```python
from build123d import *

# Parameters (mm, degrees)
SKETCH_1_W                = 499
SKETCH_1_H                = 50
EXTRUDE_1_DEPTH           = 30
CHAMFER_1_SIZE            = 3
HOLE_WIZARD_M6_1_D        = 5
HOLE_WIZARD_M6_1_DEPTH    = 15
HOLE_WIZARD_M6_1_TIP      = 1.502151548
HOLE_WIZARD_1_D           = 6.6
HOLE_WIZARD_1_DEPTH       = 30
HOLE_WIZARD_1_CBORE_D     = 11
HOLE_WIZARD_1_CBORE_DEPTH = 6.8
HOLE_WIZARD_1_TIP         = 1.982840043


with BuildPart() as part:
    # 草图1 → 凸台-拉伸1 (new body)
    with BuildSketch(Plane(origin=(0, 0, 0), x_dir=(1, 0, 0), z_dir=(0, 1, 0))):
        Rectangle(SKETCH_1_W, SKETCH_1_H)
    extrude(amount=EXTRUDE_1_DEPTH)

    # 倒角1
    chamfer_1_edges = [part.edges().sort_by_distance(p)[0] for p in [
        (249.5, 15, 25),
        (-249.5, 15, 25),
        (-249.5, 15, -25),
        (249.5, 15, -25),
    ]]
    chamfer(chamfer_1_edges, length=CHAMFER_1_SIZE)

    # M6 螺纹孔1
    with Locations(Plane(origin=(0, 30, 0), x_dir=(1, 0, 0), z_dir=(0, 1, 0))):
        with Locations((199.5, 0), (139.5, 0), (79.5, 0), (19.5, 0), (-40.5, 0), (-100.5, 0), (-160.5, 0), (-220.5, 0)):
            Hole(HOLE_WIZARD_M6_1_D / 2, depth=HOLE_WIZARD_M6_1_DEPTH)
            with Locations((0, 0, -(HOLE_WIZARD_M6_1_DEPTH + HOLE_WIZARD_M6_1_TIP / 2))):  # 118° drill point
                Cone(0, HOLE_WIZARD_M6_1_D / 2, HOLE_WIZARD_M6_1_TIP, mode=Mode.SUBTRACT)

    # 打孔尺寸(%根据)内六角圆柱头螺钉的类型1
    with Locations(Plane(origin=(0, 30, 0), x_dir=(1, 0, 0), z_dir=(0, 1, 0))):
        with Locations((169.5, 0), (49.5, 0), (-70.5, 0), (-190.5, 0)):
            CounterBoreHole(HOLE_WIZARD_1_D / 2, HOLE_WIZARD_1_CBORE_D / 2, HOLE_WIZARD_1_CBORE_DEPTH, depth=HOLE_WIZARD_1_DEPTH)
            with Locations((0, 0, -(HOLE_WIZARD_1_DEPTH + HOLE_WIZARD_1_TIP / 2))):  # 118° drill point
                Cone(0, HOLE_WIZARD_1_D / 2, HOLE_WIZARD_1_TIP, mode=Mode.SUBTRACT)


solid = part.part
```
CAD build for the part. Positions are in the model's coordinates, mm. A direction names the side the tool comes from. Coordinates: 2 decimals unless noted, no trailing zeros. Use a Markdown table: item, result. Add a question column.
(1) Which spindle directions (+Z, -Z, +X, -X, +Y, -Y) get a long thin tool onto all of the face, cutting with end or side? Do faces 1 (the face through (-3, 30, 0)), 2 (the face through (-191, 23.2, 4)). Say none if no direction does.
(2) Drill centre lines: line 1 along Z through (x, y) = (139.5, 23); line 2 along Z through (x, y) = (-190.5, 5). Where is each one in solid material? Low to high. Write a range as [from, to].
(3) Pull direction Z, two halves, no side cores. Call faces 3 (the face through (164, 27, 0)), 4 (the face through (-3, 15, 25)), 5 (the face through (-3, 15, -25)): +Z half, -Z half, draft (parallel to the pull), parting line (faces both ways), or undercut.
(4) Flat gauge pins, fed straight in: pin 1 (3 mm diameter, centred on x = 79.5, z = 0, fed in from +Y); pin 2 (4.5 mm diameter, centred on x = 199.5, z = 0, fed in from +Y); pin 3 (10.5 mm diameter, centred on x = -190.5, z = 0, fed in from -Y); pin 4 (8.5 mm diameter, centred on x = 169.5, z = 0, fed in from +Y). Where does each tip first touch, or does it go through?
Solved:
| question | item | result |
|---|---|---|
| 1 | face 1 | +Z, -Z, +X, -X, +Y |
| 1 | face 2 | +Y |
| 2 | line 1 | z = [-25, -2.5], [2.5, 25] |
| 2 | line 2 | z = [-25, -3.3], [3.3, 25] |
| 3 | face 3 | undercut |
| 3 | face 4 | +Z half |
| 3 | face 5 | -Z half |
| 4 | pin 1 | stops at y = 14.4 |
| 4 | pin 2 | stops at y = 14.85 |
| 4 | pin 3 | stops at y = 0 |
| 4 | pin 4 | stops at y = 23.2 |
